CAD build for the part. Positions are in the model's coordinates, mm. A direction names the side the tool comes from. Give positions to 0.01 mm unless a question says otherwise; leave off trailing zeros. Loops run counter-clockwise (first coordinate to the right, second up) from the corner with the lowest first, then second, coordinate; pieces in that order, holes last.
Item 1: Saw through at A-A on y = 0. Give the cut face in (x, z), plus the area to 3 significant figures.
Item 2: Saw through at B-B on x = 0. Give the cut face in (y, z).
Item 3: Drop flat-ended pins along their axis: P1, Ø12, axis at x = -49, y = 46.5, coming from the +Z side; P2, Ø2, axis at y = -12, z = 25.5, coming from the +X side; P3, Ø3, axis at y = -40.5, z = 55, coming from the -X side. Give the stop position or say it passes through.
Item 4: Saw through at C-C on z = 27.5. Give the cut face in (x, y).
Item 5: Probe probe 1 along Y at (x, z) = (0, 51); probe 2 along Y at (x, z) = (-150, 9.5); probe 3 along X at (y, z) = (15, 33.5). List the from-to ranges inside material, lowest first.
Item 6: Saw through at D-D on x = 150. Give the cut face in (y, z).
Item 7: Which spindle directions (+Z, -Z, +X, -X, +Y, -Y) get a long thin tool onto all of the face, cutting with end or side? Do faces 1 (the flat face through (156, -25, 40)), 2 (the flat face through (-125, -5, 40)), 3 (the flat face through (-58, 17, 20)). Say none if no direction does.
from build123d import *

# Parameters (mm, degrees)
LINK_PLATE_DEPTH      = 20
CENTER_BOSS_SKETCH_R  = 60
CENTER_BOSS_120_DEPTH = 50
CENTER_BORE_SKETCH_R  = 50
CENTER_BORE_100_DEPTH = 70
END_BOSS_A_SKETCH_R   = 40
END_BOSS_A_80_DEPTH   = 20
END_BOSS_B_SKETCH_R   = 40
END_BOSS_B_80_DEPTH   = 20
END_BORES_SKETCH_R    = 25
END_BORES_2X_50_DEPTH = 40


with BuildPart() as part:
    # Link Profile Sketch → Link Plate (new body)
    with BuildSketch(Plane.XY):
        with BuildLine():
            ThreePointArc((-129.642270948, 34.432003541), (-190, 0), (-129.642270948, -34.432003541))
            ThreePointArc((-129.642270948, -34.432003541), (-87.851681721, -36.458860817), (-50.548209333, -55.406484578))
            ThreePointArc((-50.548209333, -55.406484578), (5.374732367, -74.807167116), (57.949801632, -47.611138306))
            ThreePointArc((57.949801632, -47.611138306), (91.552609541, -34.039548838), (127.784288058, -33.263525714))
            ThreePointArc((127.784288058, -33.263525714), (189.977010396, -1.355964531), (130.089258317, 34.692396366))
            ThreePointArc((130.089258317, 34.692396366), (128.937737844, 34.506028192), (127.784288058, 34.331999196))
            ThreePointArc((127.784288058, 34.331999196), (85.734256685, 37.193020101), (48.597851254, 57.124853204))
            ThreePointArc((48.597851254, 57.124853204), (-0.052113987, 74.999981894), (-48.677191075, 57.057261317))
            ThreePointArc((-48.677191075, 57.057261317), (-86.6667217, 36.823333055), (-129.642270948, 34.432003541))
        make_face()
    extrude(amount=LINK_PLATE_DEPTH)

    # Center Boss Sketch → Center Boss Ø120 (add)
    with BuildSketch(Plane.XY.offset(20)):
        Circle(CENTER_BOSS_SKETCH_R)
    extrude(amount=CENTER_BOSS_120_DEPTH)

    # Center Bore Sketch → Center Bore Ø100 (cut)
    with BuildSketch(Plane.XY.offset(70)):
        Circle(CENTER_BORE_SKETCH_R)
    extrude(amount=-CENTER_BORE_100_DEPTH, mode=Mode.SUBTRACT)

    # End Boss A Sketch → End Boss A Ø80 (add)
    with BuildSketch(Plane.XY.offset(20)):
        with Locations(Location((-150, 0, 0), (0, 0, 300.593464185))):
            Circle(END_BOSS_A_SKETCH_R)
    extrude(amount=END_BOSS_A_80_DEPTH)

    # End Boss B Sketch → End Boss B Ø80 (add)
    with BuildSketch(Plane.XY.offset(20)):
        with Locations(Location((150, 0, 0), (0, 0, 236.26222597))):
            Circle(END_BOSS_B_SKETCH_R)
    extrude(amount=END_BOSS_B_80_DEPTH)

    # End Bores Sketch → End Bores 2xØ50 (cut)
    with BuildSketch(Plane.XY.offset(40)):
        with Locations((-150, 0)):
            Circle(END_BORES_SKETCH_R)
        with Locations((150, 0)):
            Circle(END_BORES_SKETCH_R)
    extrude(amount=-END_BORES_2X_50_DEPTH, mode=Mode.SUBTRACT)


solid = part.part
Results below:
1. outline: (-190, 0) - (-175, 0) - (-175, 40) - (-190, 40) - close; (-125, 0) - (-50, 0) - (-50, 70) - (-60, 70) - (-60, 20) - (-110, 20) - (-110, 40) - (-125, 40) - close; (50, 0) - (125, 0) - (125, 40) - (110, 40) - (110, 20) - (60, 20) - (60, 70) - (50, 70) - close; (175, 0) - (190, 0) - (190, 40) - (175, 40) - close
1. area: 5,800 mm2
2. outline: (-75, 0) - (-50, 0) - (-50, 70) - (-60, 70) - (-60, 20) - (-75, 20) - close; (50, 0) - (75, 0) - (75, 20) - (60, 20) - (60, 70) - (50, 70) - close
3. P1: stops at z = 20
3. P2: stops at x = 188.46
3. P3: stops at x = -45.6
4. outline: circle Ø80 at (-150, 0); circle Ø120 at (0, 0); circle Ø80 at (150, 0); hole circle Ø50 at (-150, 0); hole circle Ø100 at (0, 0); hole circle Ø50 at (150, 0)
5. probe 1: y = -60 to -50, 50 to 60
5. probe 2: y = -40 to -25, 25 to 40
5. probe 3: x = -187.08 to -170, -130 to -112.92, -58.09 to -47.7, 47.7 to 58.09, 112.92 to 130, 170 to 187.08
6. outline: (-40, 0) - (-25, 0) - (-25, 40) - (-40, 40) - close; (25, 0) - (40, 0) - (40, 40) - (25, 40) - close
7. face 1: +Z, +X, +Y, -Y
7. face 2: +Z, -X, +Y, -Y
7. face 3: +Z
